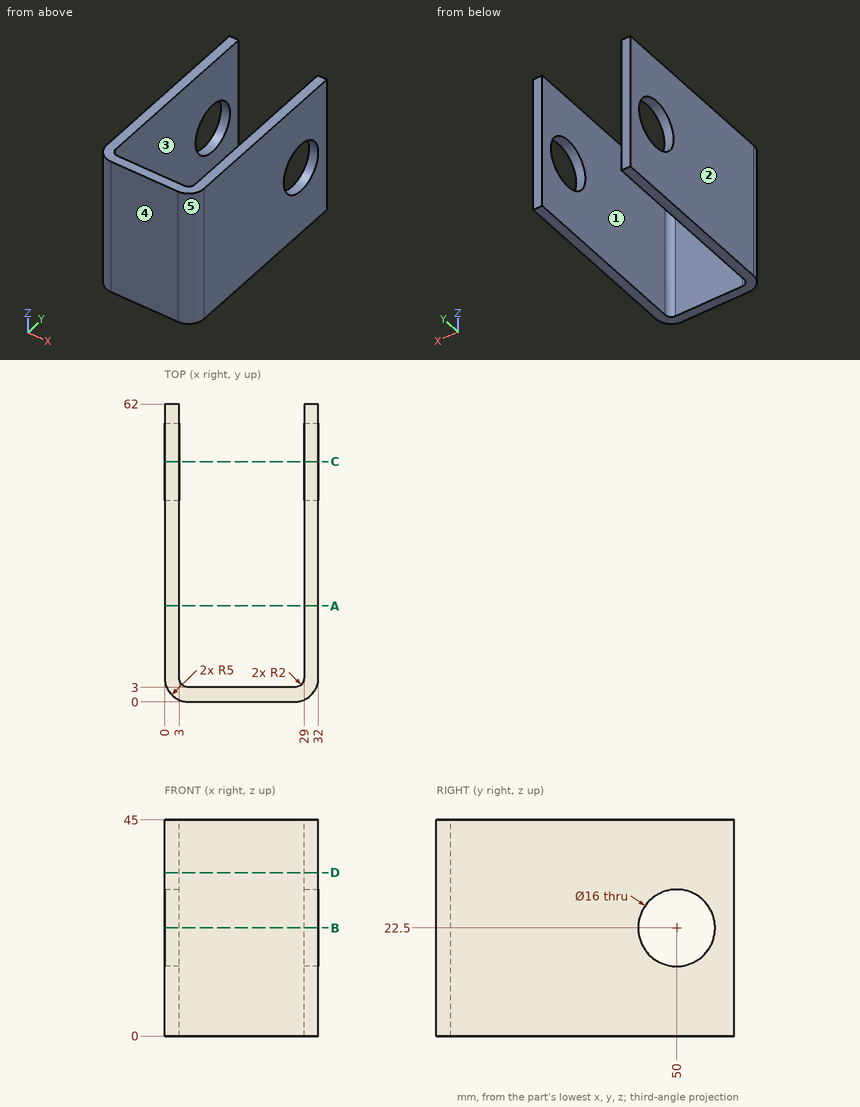
Geometry: see drawing. Coordinates: mm, zero at the bounding-box minimum. A direction names the side the tool comes from. Give positions to 0.01 mm unless a question says otherwise; leave off trailing zeros. Write each loop counter-clockwise with the first axis right and the second up, starting at its lowest first coordinate (ties: lowest second). Pieces come first, ordered by that corner, then holes. Notation, with made-up numbers: M 8.25,24.5 L 66.25,24.5 A17 cw 66.25,32.5 Z; hole C -31,-9.5 d3. An arc over 180 degrees is marked long. Answer as a JSON object with one key per item and string values.
Q1. Cut plane C-C, the plane y = 50. Return the cut outline in (x, z), then the cut area to 3 significant figures.
Geometry check:
{"outline": "M 0,0 L 3,0 L 3,14.5 L 0,14.5 Z; M 0,30.5 L 3,30.5 L 3,45 L 0,45 Z; M 29,0 L 32,0 L 32,14.5 L 29,14.5 Z; M 29,30.5 L 32,30.5 L 32,45 L 29,45 Z", "area": "174 mm^2"}
Q2. Access query for the marked faces 1 and 2. Directions: +Z, -Z, +X, -X, +Y, -Y. A direction counts if a zero-diameter tool reaches every point of the face in a straight line with its end or side. Return the directions, or none.
Geometry check:
{"face 1": "+Z, -Z, +Y", "face 2": "+Z, -Z, -X, +Y, -Y"}
Q3. Cut plane A-A, the plane y = 20. Return the cut outline in (x, z).
Geometry check:
{"outline": "M 0,0 L 3,0 L 3,45 L 0,45 Z; M 29,0 L 32,0 L 32,45 L 29,45 Z"}
Q4. Mould query, pull axis X, two halves, no side actions, for the marked faces 3, 4 and 5. Classes: +X half, -X half, draft (parallel to the pull), parting line (faces both ways), or undercut.
Geometry check:
{"face 3": "undercut", "face 4": "draft", "face 5": "+X half"}
Q5. Ray query, line 1 along X through (y, z) = (42, 11.5); line 2 along Y through (x, z) = (22, 23); line 3 along Y through (x, z) = (1.6, 22.5). Return the intervals inside material, ascending.
Geometry check:
{"line 1": "x = 0 to 3, 29 to 32", "line 2": "y = 0 to 3", "line 3": "y = 1.33 to 42, 58 to 62"}
Q6. Cut plane D-D, the plane z = 34. Return the cut outline in (x, y).
Geometry check:
{"outline": "M 0,5 A5 ccw 5,0 L 27,0 A5 ccw 32,5 L 32,62 L 29,62 L 29,5 A2 cw 27,3 L 5,3 A2 cw 3,5 L 3,62 L 0,62 Z"}
Q7. Cut plane B-B, the plane z = 22.5. Return the cut outline in (x, y), then the cut area to 3 significant figures.
Geometry check:
{"outline": "M 0,5 A5 ccw 5,0 L 27,0 A5 ccw 32,5 L 32,42 L 29,42 L 29,5 A2 cw 27,3 L 5,3 A2 cw 3,5 L 3,42 L 0,42 Z; M 0,58 L 3,58 L 3,62 L 0,62 Z; M 29,58 L 32,58 L 32,62 L 29,62 Z", "area": "345 mm^2"}
